The listing builds one solid part. Answer for the finished solid, in the listing's coordinates (mm). Face numbers are marked on the shaded views. A direction names the side the tool comes from. Round coordinates to 2 decimals unless told otherwise and drop trailing zeros. Write each loop counter-clockwise with the first axis right and the second up, starting at its lowest first coordinate (ties: lowest second). Pieces come first, ordered by that corner, then holes.
Item 1: Find section B-B on y = 149.5. Give the vertices of the cut face in (x, z).
Item 2: Find the intervals of material crossed by probe 1 along X at (y, z) = (146, 0); probe 2 along X at (y, z) = (142.25, 0); probe 3 along Y at (x, z) = (-4, 48), in increasing order.
Item 3: Find section A-A on y = 138.5. Give the vertices of the cut face in (x, z).
Item 4: Each of these flat-tipped pins is pushed along its axis until it touches: pin 1 (1 mm diameter, centred on x = -16, y = 151, fed in from +Z); pin 2 (6 mm diameter, centred on x = -35.5, y = 156.5, fed in from +Z); pin 3 (4 mm diameter, centred on y = 157.5, z = -14, fed in from -X). Where does it stop, or does it pass through?
Item 5: A tool of negligible diameter and unlimited length cuts with its end or side. For the marked faces 1, 2 and 3, from which of +Z, -Z, +X, -X, +Y, -Y can it reach the whole face along a straight path? Write none if from no direction.
Item 6: For a pull along X with two mould halves and no side action, classify the marked faces 4, 5 and 6 as +X half, -X half, draft (parallel to the pull), parting line (faces both ways), or undercut.
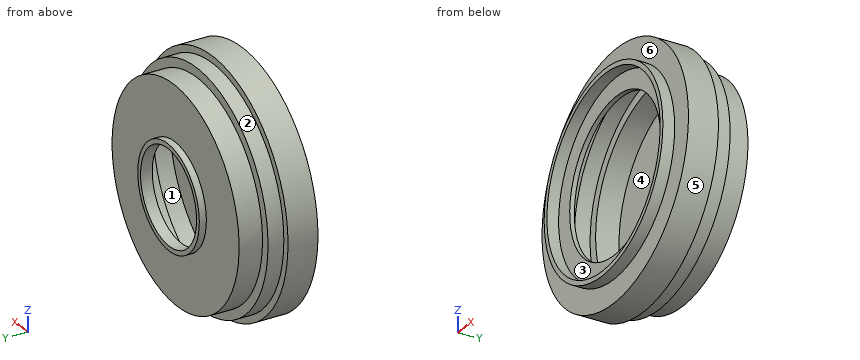
```python
from build123d import *


with BuildPart() as part:
    # Sketch1 → Revolve1 (revolve)
    with BuildSketch(Plane.XY, mode=Mode.PRIVATE) as revolve1_sk:
        Polygon((43, 136), (43, 141), (53, 141), (53, 153.772755302), (50, 153.772755302), (50, 160.531936258), (46, 160.531936258), (46, 170.5), (22.284123589, 170.5), (22.284123589, 173.5), (20.284123589, 173.5), (20.284123589, 168.5), (44, 168.5), (44, 158.531936258), (48, 158.531936258), (48, 151.772755302), (51, 151.772755302), (51, 143), (41, 143), (33, 143), (33, 141), (41, 141), (41, 136), align=None)
    revolve(revolve1_sk.sketch.rotate(Axis((0, 0, 0), (0, -1, 0)), 90), axis=Axis((0, 0, 0), (0, -1, 0)))


solid = part.part
```
Check values:
1. outline: circle Ø106 at (0, 0); hole circle Ø102 at (0, 0)
2. probe 1: x = -53 to -51, 51 to 53
2. probe 2: x = -53 to -33, 33 to 53
2. probe 3: y = 141 to 143, 151.77 to 160.53
3. outline: circle Ø86 at (0, 0); hole circle Ø82 at (0, 0)
4. pin 1: stops at z = 50.68
4. pin 2: stops at z = 40.45
4. pin 3: stops at x = -48.54
5. face 1: none
5. face 2: +Y
5. face 3: -Y
6. face 4: undercut
6. face 5: parting line
6. face 6: draft
